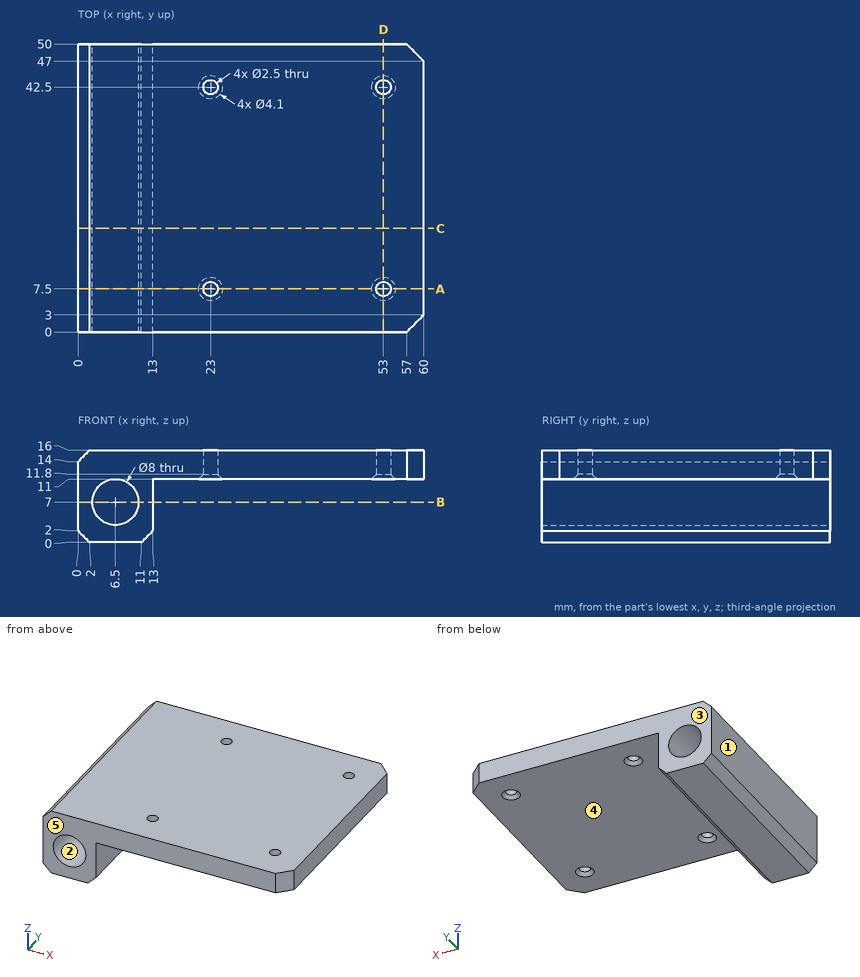
Answer from the drawing. Dimensions are ordinates in mm from the lowest x, y and z of the part. A direction names the side the tool comes from. Give positions to 0.01 mm unless a question says otherwise; leave off trailing zeros. Write each loop counter-clockwise with the first axis right and the second up, starting at its lowest first coordinate (ties: lowest second). Pieces come first, ordered by that corner, then holes. Notation, with made-up numbers: (-34, 69.25) - (-30, 69.25) arc R29 cw to (-30, 98.25) - close; hole circle Ø7 at (48.5, -23). An arc over 180 degrees is marked (long way). Answer in a Markdown table with one row per item. Add a question column.
Item 1: Section C-C, the plane y = 18 is taken. Write down the section's boundary in (x, z).
Item 2: Section B-B, the plane z = 7 is taken. Write down the section's boundary in (x, y), and give its area (3 significant figures).
Item 3: Flat-ended cylindrical pins translate along their axes: P1, Ø1, axis at y = 18.5, z = 5.5, coming from the +X side; P2, Ø23.5, axis at x = 25, y = 13.5, coming from the -Z side; P3, Ø1.5, axis at x = 53, y = 7.5, coming from the +Z side; P4, Ø3, axis at x = 23, y = 7.5, coming from the -Z side. Find the tip coordinate at first contact, or state that the pin passes through.
Item 4: Section A-A, the plane y = 7.5 is taken. Write down the section's boundary in (x, z).
Item 5: A tool of negligible diameter and unlimited length cuts with its end or side. For the marked faces 4 and 5, from which of +Z, -Z, +X, -X, +Y, -Y can it reach the whole face along a straight path? Write none if from no direction.
Item 6: Section D-D, the plane x = 53 is taken. Write down the section's boundary in (y, z), and give its area (3 significant figures).
Item 7: Find the intervals of material crossed by L1, parallel to Y at x = 23, z = 14.85; L2, parallel to X at y = 20, z = 7; L3, parallel to Z at x = 21, y = 14, in increasing order.
Item 8: Determine the mould class of the marked faces 1, 2 and 3 for opening direction X: pulls with the +X half, pulls with the -X half, needs draft (parallel to the pull), parting line crosses it, or undercut.
Recorded:
| question | item | result |
|---|---|---|
| 1 | outline | (0, 2) - (2, 0) - (11, 0) - (13, 2) - (13, 11) - (60, 11) - (60, 16) - (2, 16) - (0, 14) - close; hole circle Ø8 at (6.5, 7) |
| 2 | outline | (0, 0) - (2.5, 0) - (2.5, 50) - (0, 50) - close; (10.5, 0) - (13, 0) - (13, 50) - (10.5, 50) - close |
| 2 | area | 250 mm2 |
| 3 | P1 | stops at x = 13 |
| 3 | P2 | stops at z = 11 |
| 3 | P3 | passes through |
| 3 | P4 | stops at z = 11.55 |
| 4 | outline | (0, 2) - (2, 0) - (11, 0) - (13, 2) - (13, 11) - (20.95, 11) - (21.75, 11.8) - (21.75, 16) - (2, 16) - (0, 14) - close; (24.25, 11.8) - (25.05, 11) - (50.95, 11) - (51.75, 11.8) - (51.75, 16) - (24.25, 16) - close; (54.25, 11.8) - (55.05, 11) - (60, 11) - (60, 16) - (54.25, 16) - close; hole circle Ø8 at (6.5, 7) |
| 5 | face 4 | -Z, +X, +Y, -Y |
| 5 | face 5 | +Z, -Z, +X, -X, -Y |
| 6 | outline | (0, 11) - (5.45, 11) - (6.25, 11.8) - (6.25, 16) - (0, 16) - close; (8.75, 11.8) - (9.55, 11) - (40.45, 11) - (41.25, 11.8) - (41.25, 16) - (8.75, 16) - close; (43.75, 11.8) - (44.55, 11) - (50, 11) - (50, 16) - (43.75, 16) - close |
| 6 | area | 224 mm2 |
| 7 | L1 | y = 0 to 6.25, 8.75 to 41.25, 43.75 to 50 |
| 7 | L2 | x = 0 to 2.5, 10.5 to 13 |
| 7 | L3 | z = 11 to 16 |
| 8 | face 1 | pulls with the -X half |
| 8 | face 2 | undercut |
| 8 | face 3 | needs draft |
